Check sheet for the modelled part. Datum: model origin and axes. Units: mm. Give positions to 0.01 mm unless a question says otherwise; leave off trailing zeros. Write each loop counter-clockwise with the first axis right and the second up, starting at its lowest first coordinate (ties: lowest second). Pieces come first, ordered by that corner, then holes. Notation, with made-up numbers: M 22,73.25 L 77,73.25 A23 cw 77,108.25 Z; hole C 69.5,72.5 d10. An arc over 180 degrees is marked long. Write item = value, one per line. Start each with the question number.
1) Go/stop test with flat-tipped pins: pin 1 (1.5 mm diameter, centred on y = 10, z = 4, fed in from -X); pin 2 (1.5 mm diameter, centred on y = -112, z = 3, fed in from +X). Record where each tip stops, or that it passes through.
2) Mould release check, pull along Y, two halves, no side actions. Record for faces 1 (the cylindrical face through (0.8, 141.2, 3.9)), 2 (the cylindrical face through (-134.91, -103.44, 3.94)), 3 (the flat face through (-2, 2, 0)), 4 (the cylindrical face through (0.8, -128.8, 3.9)): released by +Y, released by -Y, zero draft, split by the parting line, or undercut.
3) Cross-section at C-C, the plane z = 3. Record the cut outline in (x, y) (3 decimals), plus the area to 3 significant figures.
4) Cross-section at B-B, the plane y = -67.5. Record the cut outline in (x, z), plus the area to 3 significant figures.
5) Cross-section at A-A, the plane x = 0. Record the cut outline in (y, z) (3 decimals).
6) Cross-section at D-D, the plane y = 135. Record the cut outline in (x, z), plus the area to 3 significant figures.
7) Scan lines: line 1 along Y through (x, z) = (0, 4) (3 decimals); line 2 along X through (y, z) = (65, 4.5); line 3 along Y through (x, z) = (-112.5, 4). Record each from-to range of solid material in increasing order. Write a range as [from, to].
```python
from build123d import *

# Parameters (mm, degrees)
SKETCH1_R           = 170
BOSS_EXTRUDE1_DEPTH = 8
SKETCH3_R           = 6.25
CUT_EXTRUDE1_DEPTH  = 10
SKETCH4_R           = 5.125
CUT_EXTRUDE2_DEPTH  = 10


with BuildPart() as part:
    # Sketch1 → Boss-Extrude1 (new body)
    with BuildSketch(Plane.XY):
        Circle(SKETCH1_R)
    extrude(amount=BOSS_EXTRUDE1_DEPTH)

    # Sketch3 → Cut-Extrude1 (cut)
    with BuildSketch(Plane(origin=(0, 0, 0), x_dir=(-1, 0, 0), z_dir=(0, 0, -1))):
        with Locations((116.913429511, 67.5)):
            Circle(SKETCH3_R)
        with Locations((0, 135)):
            Circle(SKETCH3_R)
        with Locations((116.913429511, -67.5)):
            Circle(SKETCH3_R)
        with Locations((0, -135)):
            Circle(SKETCH3_R)
        with Locations((-116.913429511, -67.5)):
            Circle(SKETCH3_R)
        with Locations((-116.913429511, 67.5)):
            Circle(SKETCH3_R)
    extrude(amount=-CUT_EXTRUDE1_DEPTH, mode=Mode.SUBTRACT)

    # Sketch4 → Cut-Extrude2 (cut)
    with BuildSketch(Plane(origin=(0, 0, 0), x_dir=(-1, 0, 0), z_dir=(0, 0, -1))):
        with Locations((0, 80)):
            Circle(SKETCH4_R)
    extrude(amount=-CUT_EXTRUDE2_DEPTH, mode=Mode.SUBTRACT)


solid = part.part
```
Reply:
q1.pin_1 = -169.75
q1.pin_2 = 128.54
q2.face_1 = undercut
q2.face_2 = split by the parting line
q2.face_3 = zero draft
q2.face_4 = undercut
q3.outline = C 0,0 d340; hole C -116.913,-67.5 d12.5; hole C -116.913,67.5 d12.5; hole C 0,-135 d12.5; hole C 0,135 d12.5; hole C 0,80 d10.25; hole C 116.913,-67.5 d12.5; hole C 116.913,67.5 d12.5
q3.area = 90,000 mm2
q4.outline = M -156.02,0 L -123.16,0 L -123.16,8 L -156.02,8 Z; M -110.66,0 L 110.66,0 L 110.66,8 L -110.66,8 Z; M 123.16,0 L 156.02,0 L 156.02,8 L 123.16,8 Z
q4.area = 2,300 mm2
q5.outline = M -170,0 L -141.25,0 L -141.25,8 L -170,8 Z; M -128.75,0 L 74.875,0 L 74.875,8 L -128.75,8 Z; M 85.125,0 L 128.75,0 L 128.75,8 L 85.125,8 Z; M 141.25,0 L 170,0 L 170,8 L 141.25,8 Z
q6.outline = M -103.32,0 L -6.25,0 L -6.25,8 L -103.32,8 Z; M 6.25,0 L 103.32,0 L 103.32,8 L 6.25,8 Z
q6.area = 1,550 mm2
q7.line_1 = [-170, -141.25], [-128.75, 74.875], [85.125, 128.75], [141.25, 170]
q7.line_2 = [-157.08, -122.64], [-111.19, 111.19], [122.64, 157.08]
q7.line_3 = [-127.45, -71.93], [-63.07, 63.07], [71.93, 127.45]
